from build123d import *

# Parameters (mm, degrees)
SKETCH_1_W      = 60
SKETCH_1_H      = 102
SKETCH_1_R      = 2.25
EXTRUDE_1_DEPTH = 5
SKETCH_2_W      = 52
SKETCH_2_H      = 80
EXTRUDE_2_DEPTH = 75
SKETCH_3_R      = 5
EXTRUDE_3_DEPTH = 12
EXTRUDE_3_TAPER = 5
FILLET_1_R      = 1
SKETCH_4_W      = 14
SKETCH_4_H      = 72
EXTRUDE_4_DEPTH = 12


with BuildPart() as part:
    # 草图1 → 凸台-拉伸1 (new body)
    with BuildSketch(Plane.XY):
        Rectangle(SKETCH_1_W, SKETCH_1_H)
        with Locations((0, 45.563491435)):
            Circle(SKETCH_1_R, mode=Mode.SUBTRACT)
        with Locations((0, -44.436508565)):
            Circle(SKETCH_1_R, mode=Mode.SUBTRACT)
    extrude(amount=EXTRUDE_1_DEPTH)

    # 草图2 → 凸台-拉伸2 (add)
    with BuildSketch(Plane(origin=(0, 0, 0), x_dir=(-1, 0, 0), z_dir=(0, 0, -1))):
        Rectangle(SKETCH_2_W, SKETCH_2_H)
    extrude(amount=EXTRUDE_2_DEPTH)

    # 草图3 → 凸台-拉伸3 (add)
    with BuildSketch(Plane.XY.offset(5)):
        with Locations((10, -23)):
            Circle(SKETCH_3_R)
    extrude(amount=EXTRUDE_3_DEPTH, taper=EXTRUDE_3_TAPER)

    # 圆角1
    fillet_1_edges = [part.edges().sort_by_distance(p)[0] for p in [
        (30, -51, 2.5),
        (-30, -51, 2.5),
        (-30, 51, 2.5),
        (30, 51, 2.5),
    ]]
    fillet(fillet_1_edges, radius=FILLET_1_R)

    # 草图4 → 凸台-拉伸4 (add)
    with BuildSketch(Plane(origin=(0, 0, -75), x_dir=(-1, 0, 0), z_dir=(0, 0, -1))):
        with Locations((15, 0)):
            Rectangle(SKETCH_4_W, SKETCH_4_H)
    extrude(amount=EXTRUDE_4_DEPTH)


solid = part.part
Source: CAD feature listing. Evaluate the final solid. Frame: model axes, mm. A direction names the side the tool comes from. Give positions to 0.01 mm unless a question says otherwise; leave off trailing zeros. Write each loop counter-clockwise with the first axis right and the second up, starting at its lowest first coordinate (ties: lowest second). Pieces come first, ordered by that corner, then holes. Notation, with made-up numbers: M 51.25,46.25 L 94.25,46.25 A25 cw 94.25,71.25 Z; hole C -36.5,-21 d7. An arc over 180 degrees is marked long. Return JSON: item names as keys, results as strings. Group by question number.
1) Cut plane D-D, the plane z = -29. Output: boundary loops of the cut face in (x, y).
2) Cut plane C-C, the plane y = -33.5. Output: boundary loops of the cut face in (x, z).
3) Set-up query: faces 1 (the face through (30, -1, 2)), 2 (the face through (-15, -36, -81)), 3 (the face through (-22, -1, -81)), 4 (the face through (-15, 36, -81)), 5 (the face through (26, -1, -37)). Return all of +Z, -Z, +X, -X, +Y, -Y with unobstructed straight access to the full face (end or side cutting, diameter ignored); none if empty.
4) Draft query along Y for faces 6 (the face through (-8, -1, -81)), 7 (the face through (-0.488, -46.633, 2.465)), 8 (the face through (-0.488, 43.367, 2.465)), 9 (the face through (0, -40, -37)). Return one class per face: released by +Y, released by -Y, zero draft, split by the parting line, or undercut.
5) Cut plane A-A, the plane x = 0. Output: boundary loops of the cut face in (y, z), then the cut area to 4 significant figures.
6) Cut plane B-B, the plane x = 10. Output: boundary loops of the cut face in (y, z), then the cut area to 3 significant figures.
7) First-contact query: pin 1 Ø13 at (y, z) = (-8, -79) entering from +X; pin 2 Ø7 at (x, y) = (0, -44.44) entering from +Z; pin 3 Ø2 at (y, z) = (8, -2) entering from -X. Flat tips, straight axial feed; report the tip coordinate or a pass-through.
8) Ray query, L1, parallel to Z at x = -10.5, y = -29; L2, parallel to Y at x = -21.5, z = -27; L3, parallel to Z at x = 27, y = 47. Return the intervals inside material, ascending.
Data:
{
 "1": {"outline": "M -26,-40 L 26,-40 L 26,40 L -26,40 Z"},
 "2": {"outline": "M -30,0 L -26,0 L -26,-75 L -22,-75 L -22,-87 L -8,-87 L -8,-75 L 26,-75 L 26,0 L 30,0 L 30,5 L -30,5 Z"},
 "3": {"face 1": "+Z, -Z, +X, +Y, -Y", "face 2": "-Z, +X, -X, -Y", "face 3": "-Z, -X, +Y, -Y", "face 4": "-Z, +X, -X, +Y", "face 5": "-Z, +X, +Y, -Y"},
 "4": {"face 6": "zero draft", "face 7": "undercut", "face 8": "undercut", "face 9": "released by -Y"},
 "5": {"outline": "M -51,0 L -46.69,0 L -46.69,5 L -51,5 Z; M -42.19,0 L -40,0 L -40,-75 L 40,-75 L 40,0 L 43.31,0 L 43.31,5 L -42.19,5 Z; M 47.81,0 L 51,0 L 51,5 L 47.81,5 Z", "area": "6,465 mm²"},
 "6": {"outline": "M -51,0 L -40,0 L -40,-75 L 40,-75 L 40,0 L 51,0 L 51,5 L -18,5 L -19.05,17 L -26.95,17 L -28,5 L -51,5 Z", "area": "6,620 mm²"},
 "7": {"pin 1": "stops at x = 26", "pin 2": "stops at z = 5", "pin 3": "stops at x = -26"},
 "8": {"L1": "z = -87 to 5", "L2": "y = -40 to 40", "L3": "z = 0 to 5"}
}
